Geometry check sheet. Reference: drawing and pictorial views, mm from the part's lowest x, y, z. A direction names the side the tool comes from. Coordinates: 2 decimals unless noted, no trailing zeros. Write each loop counter-clockwise with the first axis right and the second up, starting at its lowest first coordinate (ties: lowest second). Pieces come first, ordered by that corner, then holes.
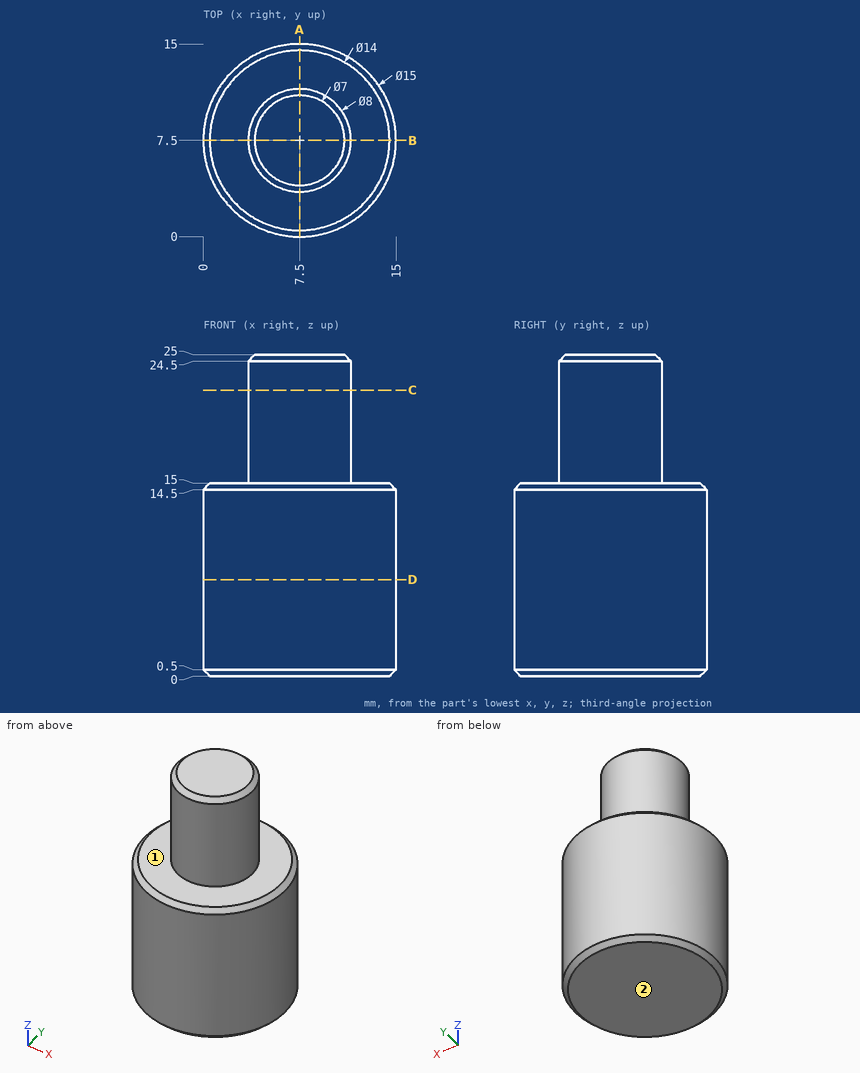
1. Sectioned sample at C-C, the plane z = 22.25. Record the boundary of the cut face in (x, y), and give its area (3 significant figures).
2. Material ranges on L1, parallel to Z at x = 11.25, y = 6; L2, parallel to Y at x = 7.5, z = 18.75; L3, parallel to X at y = 9.25, z = 3, recorded low to high.
3. Sectioned sample at D-D, the plane z = 7.5. Record the boundary of the cut face in (x, y), and give its area (3 significant figures).
4. Sectioned sample at A-A, the plane x = 7.5. Record the boundary of the cut face in (y, z).
5. Tool access check on the marked faces 1 and 2. Record the directions out of +Z, -Z, +X, -X, +Y, -Y that give a thin tool (end or side, any length) a straight path to the whole face; none if there is none.
6. Gauge pin test, flat ends, axial feed: P1, Ø6, axis at y = 11.5, z = 3, coming from the +X side; P2, Ø1, axis at x = 7, y = 2, coming from the +Z side; P3, Ø4, axis at y = 2.5, z = 3, coming from the -X side. Record the tip position at first contact, or that the pin passes through.
Outcome:
1. outline: circle Ø8 at (7.5, 7.5)
1. area: 50.3 mm2
2. L1: z = 0 to 15
2. L2: y = 3.5 to 11.5
2. L3: x = 0.21 to 14.79
3. outline: circle Ø15 at (7.5, 7.5)
3. area: 177 mm2
4. outline: (0, 0.5) - (0.5, 0) - (14.5, 0) - (15, 0.5) - (15, 14.5) - (14.5, 15) - (11.5, 15) - (11.5, 24.5) - (11, 25) - (4, 25) - (3.5, 24.5) - (3.5, 15) - (0.5, 15) - (0, 14.5) - close
5. face 1: +Z
5. face 2: -Z, +X, -X, +Y, -Y
6. P1: stops at x = 14.93
6. P2: stops at z = 15
6. P3: stops at x = 0.63
